from build123d import *

# Parameters (mm, degrees)
MOUNT_SIDE_PROFILE_SKETCH_R            = 50
MOUNT_SIDE_PROFILE_SKETCH_R_2          = 32.5
CLAMP_COLLAR_BODY_DEPTH                = 37.5
BASE_PLATE_SKETCH_R                    = 37.5
BASE_PLATE_15MM_DEPTH                  = 15
SOCKET_BOSS_SKETCH_R                   = 27.5
SOCKET_BOSS_DEPTH                      = 55
SKETCH10_3_R                           = 25
SOCKET_BOSS_RELIEF_CUT_DEPTH           = 5
SOCKET_START                           = -55
SKETCH10_4_R                           = 15
SOCKET_BORE_DEPTH                      = 50
SOCKET_COUNTERBORE_SKETCH_40_R         = 20
SOCKET_COUNTERBORE_40_DEPTH            = 5
CURVED_ARM_DEPTH                       = 37.5
PIPE_BORE_CUT_DEPTH                    = 291.839302709
PIPE_BORE_CUT_DEPTH_BACK               = 291.839302709
SKETCH1_2_R                            = 32.5
ARM_RIB_20MM_DEPTH                     = 10
ARM_WEB_30MM_DEPTH                     = 15
CLAMP_LUG_DEPTH                        = 35
CLAMP_SPLIT_SLOT_DEPTH                 = 2.5
CLAMP_BOLT_HOLE_CBORE_13_5_D           = 13.5
CLAMP_BOLT_HOLE_CBORE_13_5_CBORE_D     = 22
CLAMP_BOLT_HOLE_CBORE_13_5_CBORE_DEPTH = 6.6


with BuildPart() as part:
    # Mount Side Profile Sketch → Clamp Collar Body (new, symmetric)
    with BuildSketch(Plane.XY):
        with Locations((0, 145)):
            Circle(MOUNT_SIDE_PROFILE_SKETCH_R)
        with Locations((0, 145)):
            Circle(MOUNT_SIDE_PROFILE_SKETCH_R_2, mode=Mode.SUBTRACT)
    extrude(amount=CLAMP_COLLAR_BODY_DEPTH, both=True)



with BuildPart() as body_2:
    # Base Plate Sketch → Base Plate 15mm (new body)
    with BuildSketch(Plane(origin=(0, 0, 0), x_dir=(1, 0, 0), z_dir=(0, 1, 0))):
        with Locations(Location((-175, 0, 0), (0, 0, 270))):
            Circle(BASE_PLATE_SKETCH_R)
    extrude(amount=BASE_PLATE_15MM_DEPTH)

    # Socket Boss Sketch → Socket Boss (add)
    with BuildSketch(Plane.XZ):
        with Locations(Location((-175, 0, 0), (0, 0, 270))):
            Circle(SOCKET_BOSS_SKETCH_R)
    extrude(amount=-SOCKET_BOSS_DEPTH)

    # Sketch10_3 → Socket Boss Relief Cut (cut)
    with BuildSketch(Plane.XZ):
        with Locations(Location((-175, 0, 0), (0, 0, 270))):
            Circle(SKETCH10_3_R)
    extrude(amount=-SOCKET_BOSS_RELIEF_CUT_DEPTH, mode=Mode.SUBTRACT)

    # Sketch10_4 → Socket Bore (cut)
    with BuildSketch(Plane.XZ.offset(SOCKET_START)):
        with Locations(Location((-175, 0, 0), (0, 0, 270))):
            Circle(SKETCH10_4_R)
    extrude(amount=SOCKET_BORE_DEPTH, mode=Mode.SUBTRACT)

    # Socket Counterbore Sketch _40 → Socket Counterbore _40 (cut)
    with BuildSketch(Plane(origin=(0, 55, 0), x_dir=(1, 0, 0), z_dir=(0, 1, 0))):
        with Locations(Location((-175, 0, 0), (0, 0, 270))):
            Circle(SOCKET_COUNTERBORE_SKETCH_40_R)
    extrude(amount=-SOCKET_COUNTERBORE_40_DEPTH, mode=Mode.SUBTRACT)


with BuildPart() as part_1:
    add(part.part)

    add(body_2.part)  # Curved Arm merges body 2
    # Curved Arm Profile Sketch → Curved Arm (add, symmetric)
    with BuildSketch(Plane.XY):
        with BuildLine():
            Line((-175, 0), (-30, 0))
            ThreePointArc((-30, 0), (26.568542495, 23.431457505), (50, 80))
            Line((50, 80), (50, 145))
            ThreePointArc((50, 145), (-46.097722286, 164.364916731), (35, 109.292857857))
            Line((35, 109.292857857), (35, 80))
            ThreePointArc((35, 80), (15.961940777, 34.038059223), (-30, 15))
            Line((-30, 15), (-175, 15))
            Line((-175, 15), (-175, 0))
        make_face()
    extrude(amount=CURVED_ARM_DEPTH, both=True)

    # Sketch1_2 → Pipe Bore Cut (cut, two sides: drawn at the far end of the back side and taken through both)
    with BuildSketch(Plane.XY.offset(-PIPE_BORE_CUT_DEPTH_BACK)):
        with Locations((0, 145)):
            Circle(SKETCH1_2_R)
    extrude(amount=PIPE_BORE_CUT_DEPTH + PIPE_BORE_CUT_DEPTH_BACK, mode=Mode.SUBTRACT)

    # Sketch12_3 → Arm Rib 20mm (add, symmetric)
    with BuildSketch(Plane.XY):
        with BuildLine():
            Line((-151.5, 35), (-151.5, 15))
            Line((-151.5, 15), (-30, 15))
            ThreePointArc((-30, 15), (15.961940777, 34.038059223), (35, 80))
            Line((35, 80), (35, 109.292857857))
            ThreePointArc((35, 109.292857857), (0, 95), (-35, 109.292857857))
            Line((-35, 109.292857857), (-35, 90))
            ThreePointArc((-35, 90), (-51.109127035, 51.109127035), (-90, 35))
            Line((-90, 35), (-151.5, 35))
        make_face()
    extrude(amount=ARM_RIB_20MM_DEPTH, both=True)

    # Sketch12_4 → Arm Web 30mm (add, symmetric)
    with BuildSketch(Plane.XY):
        with BuildLine():
            Line((-151.5, 50), (-151.5, 35))
            Line((-151.5, 35), (-90, 35))
            ThreePointArc((-90, 35), (-51.109127035, 51.109127035), (-35, 90))
            Line((-35, 90), (-35, 109.292857857))
            ThreePointArc((-35, 109.292857857), (-46.097722286, 125.635083269), (-50, 145))
            Line((-50, 145), (-50, 90))
            ThreePointArc((-50, 90), (-61.715728753, 61.715728753), (-90, 50))
            Line((-90, 50), (-151.5, 50))
        make_face()
    extrude(amount=ARM_WEB_30MM_DEPTH, both=True)

    # Clamp Lug Sketch → Clamp Lug (add, symmetric)
    with BuildSketch(Plane(origin=(0, 0, 0), x_dir=(0, 0, -1), z_dir=(1, 0, 0))):
        with BuildLine():
            Line((19.923893962, 206.743114855), (22.482334998, 177.5))
            Line((22.482334998, 177.5), (-22.482334998, 177.5))
            Line((-22.482334998, 177.5), (-19.923893962, 206.743114855))
            ThreePointArc((-19.923893962, 206.743114855), (0, 225), (19.923893962, 206.743114855))
        make_face()
    extrude(amount=CLAMP_LUG_DEPTH, both=True)

    # Clamp Split Slot Sketch → Clamp Split Slot (cut, symmetric)
    with BuildSketch(Plane(origin=(0, 0, 0), x_dir=(0, 0, -1), z_dir=(1, 0, 0))):
        with BuildLine():
            Line((-37.855398527, 208.311918224), (-41.845299437, 162.707142143))
            Line((-41.845299437, 162.707142143), (41.845299437, 162.707142143))
            Line((41.845299437, 162.707142143), (37.855398527, 208.311918224))
            ThreePointArc((37.855398527, 208.311918224), (0, 243), (-37.855398527, 208.311918224))
        make_face()
    extrude(amount=CLAMP_SPLIT_SLOT_DEPTH, both=True, mode=Mode.SUBTRACT)

    # Clamp Bolt Hole CBore _13.5 (through all)
    with Locations(Plane.ZY.offset(35)):
        with Locations((0, 205)):
            CounterBoreHole(CLAMP_BOLT_HOLE_CBORE_13_5_D / 2, CLAMP_BOLT_HOLE_CBORE_13_5_CBORE_D / 2, CLAMP_BOLT_HOLE_CBORE_13_5_CBORE_DEPTH)


solid = part_1.part
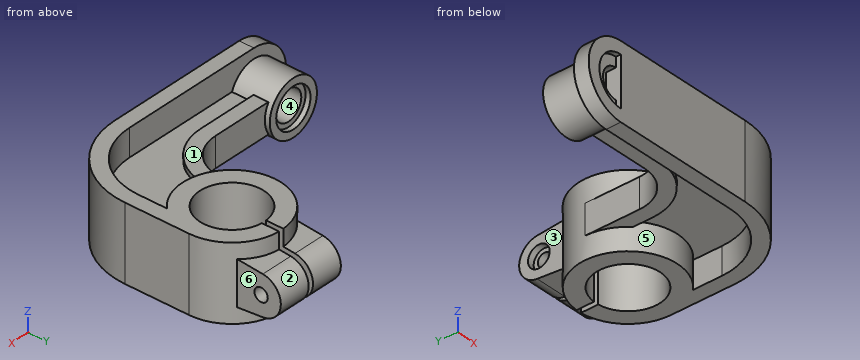
Geometry check sheet. Reference: the model listing, model coordinates, mm. Face numbers are marked on the shaded views. A direction names the side the tool comes from. Give positions to 0.01 mm unless a question says otherwise; leave off trailing zeros. Write each loop counter-clockwise with the first axis right and the second up, starting at its lowest first coordinate (ties: lowest second). Pieces come first, ordered by that corner, then holes. Notation, with made-up numbers: (29, 81) - (75, 81) arc R15 ccw to (75, 85) - close; hole circle Ø3 at (19, 63.25). An arc over 180 degrees is marked (long way). Put each result on its own line as item: value.
1. Draft check along Y on the marked faces 1, 2 and 3. Enter one of: +Y half, -Y half, draft (parallel to the pull), parting line (faces both ways), or undercut.
Ans:
face 1: undercut
face 2: +Y half
face 3: draft
2. Sectioned sample at A-A, the plane y = 134. Enter the section's corners in (x, z) (3 decimals).
Ans:
outline: (-50, -15) - (-48.775, -15) - (-48.775, -37.5) - (-30.582, -37.5) - (-30.582, 37.5) - (-48.775, 37.5) - (-48.775, 15) - (-50, 15) - close; (30.582, -37.5) - (50, -37.5) - (50, 37.5) - (30.582, 37.5) - close
3. Sectioned sample at B-B, the plane x = -23.5. Enter the section's corners in (y, z), plus the area to 3 significant figures.
Ans:
outline: (0.26, -37.5) - (15.33, -37.5) - (15.33, -10) - (100.87, -10) - (100.87, -37.5) - (122.55, -37.5) - (122.55, 37.5) - (100.87, 37.5) - (100.87, 10) - (15.33, 10) - (15.33, 37.5) - (0.26, 37.5) - close; (167.45, -37.5) - (189.13, -37.5) - (189.13, -21.46) - (206.74, -19.92) arc R20 ccw to (206.74, 19.92) - (189.13, 21.46) - (189.13, 37.5) - (167.45, 37.5) - close; hole circle Ø13.5 at (205, 0)
area: 7,240 mm²
4. Set-up check for the marked faces 4, 5 and 6: record each of +Z, -Z, +X, -X, +Y, -Y from which the full face is reachable in a straight line by a thin tool's end or side.
Ans:
face 4: +Y
face 5: none
face 6: +Z, -Z, +X, +Y
5. Thickness scan on line 1 (Y direction, x = 16.5, z = 0); line 2 (Y direction, x = -5.5, z = 23); line 3 (Y direction, x = -118, z = 7). Record the ranges inside material, lowest first.
Ans:
line 1: y = 14.9 to 117, 173 to 198.25, 211.75 to 225
line 2: y = 3.84 to 19.79, 95.3 to 112.97, 177.03 to 194.7
line 3: y = 0 to 50
6. Go/stop test with flat-tipped pins: pin 1 (10 mm diameter, centred on x = -143, z = -18.5, fed in from +Y); pin 2 (12 mm diameter, centred on y = 76, z = 5, fed in from +X); pin 3 (12.5 mm diameter, centred on x = -184, z = -10.5, fed in from -Y); pin 4 (5 mm diameter, centred on x = 15.5, y = 87.5, fed in from -Z). Record where each tip stops, or that it passes through.
Ans:
pin 1: stops at y = 50
pin 2: stops at x = 50
pin 3: stops at y = 5
pin 4: stops at z = -10
7. Sectioned sample at C-C, the plane x = -135. Enter the section's corners in (y, z), plus the area to 4 significant figures.
Ans:
outline: (0, -37.5) - (15, -37.5) - (15, -10) - (35, -10) - (35, -15) - (50, -15) - (50, 15) - (35, 15) - (35, 10) - (15, 10) - (15, 37.5) - (0, 37.5) - close
area: 1,975 mm²
8. Sectioned sample at D-D, the plane y = 83.5. Enter the section's corners in (x, z), plus the area to 3 significant figures.
Ans:
outline: (-50.53, -15) - (-35.39, -15) - (-35.39, -10) - (35, -10) - (35, -37.5) - (50, -37.5) - (50, 37.5) - (35, 37.5) - (35, 10) - (-35.39, 10) - (-35.39, 15) - (-50.53, 15) - close
area: 2,990 mm²
